Geometry check sheet. Reference: the model listing, model coordinates, mm. Face numbers are marked on the shaded views. A direction names the side the tool comes from. Coordinates: 2 decimals unless noted, no trailing zeros. Loops run counter-clockwise (first coordinate to the right, second up) from the corner with the lowest first, then second, coordinate; pieces in that order, holes last. Notation, with made-up numbers: (77, 41) - (109, 41) arc R25 cw to (109, 65) - close; hole circle Ø10 at (85.25, 3). An arc over 180 degrees is marked (long way). Write each question's results on one line, items separated by ' | '. Start each with the question number.
(1) Sectioned sample at C-C (y = 11.5). Enter the section's corners in (x, z), plus the area to 4 significant figures.
(2) Sectioned sample at D-D (x = -5.5). Enter the section's corners in (y, z), plus the area to 3 significant figures.
(3) Sectioned sample at B-B (z = 0). Enter the section's corners in (x, y), plus the area to 4 significant figures.
(4) Access from +Z, -Z, +X, -X, +Y, -Y to the whole of each face (thin tool, end or side, straight path). Record for the marked faces 4, 5 and 6.
(5) Go/stop test with flat-tipped pins: pin 1 Ø7.5 at (x, z) = (-3, 1.5) entering from -Y; pin 2 Ø4.5 at (x, z) = (0, 32.5) entering from -Y. Record where each tip stops, or that it passes through.
(6) Mould release check, pull along Z, two halves, no side actions. Record for the marked faces 1, 2 and 3: pulls with the +Z half, pulls with the -Z half, needs draft (parallel to the pull), parting line crosses it, or undercut.
(7) Sectioned sample at A-A (y = -34.5). Enter the section's corners in (x, z).
(8) Material ranges on probe 1 along Y at (x, z) = (6.2, 0); probe 2 along X at (y, z) = (-37, -20); probe 3 along Y at (x, z) = (-3.5, 0), recorded low to high.
from build123d import *

# Parameters (mm, degrees)
SKETCH1_R             = 27.5
BOSS_EXTRUDE2_DEPTH   = 7.5
M6_TAPPED_HOLE1_D     = 5
M6_TAPPED_HOLE1_DEPTH = 17
M6_TAPPED_HOLE1_TIP   = 1.502151548
BOSS_EXTRUDE3_START   = -2
SKETCH5_R             = 27.5
SKETCH5_R_2           = 26
BOSS_EXTRUDE3_DEPTH   = 2
CHAMFER1_SIZE         = 5
SKETCH4_R             = 2.5
CUT_EXTRUDE1_DEPTH    = 15
CHAMFER2_SIZE         = 1
CHAMFER3_SIZE         = 0.5


with BuildPart() as part:
    # Sketch1 → Boss-Extrude2 (new, symmetric)
    with BuildSketch(Plane(origin=(0, 0, 0), x_dir=(0, 0, -1), z_dir=(1, 0, 0))):
        with BuildLine():
            Line((-37.5, -42.5), (-12.5, -42.5))
            Line((-12.5, -42.5), (-12.5, -32.5))
            ThreePointArc((-12.5, -32.5), (-11.035533906, -28.964466094), (-7.5, -27.5))
            Line((-7.5, -27.5), (7.5, -27.5))
            ThreePointArc((7.5, -27.5), (11.035533906, -28.964466094), (12.5, -32.5))
            Line((12.5, -32.5), (12.5, -42.5))
            Line((12.5, -42.5), (37.5, -42.5))
            Line((37.5, -42.5), (37.5, 42.5))
            Line((37.5, 42.5), (-37.5, 42.5))
            Line((-37.5, 42.5), (-37.5, -42.5))
        make_face()
        with Locations((0, 11.5)):
            Circle(SKETCH1_R, mode=Mode.SUBTRACT)
    extrude(amount=BOSS_EXTRUDE2_DEPTH, both=True)

    # M6 Tapped Hole1
    with Locations(Plane(origin=(0, -42.5, 0), x_dir=(-1, 0, 0), z_dir=(0, -1, 0))):
        with Locations((0, -32.5), (0, 32.5)):
            Hole(M6_TAPPED_HOLE1_D / 2, depth=M6_TAPPED_HOLE1_DEPTH)
            with Locations((0, 0, -(M6_TAPPED_HOLE1_DEPTH + M6_TAPPED_HOLE1_TIP / 2))):  # 118° drill point
                Cone(0, M6_TAPPED_HOLE1_D / 2, M6_TAPPED_HOLE1_TIP, mode=Mode.SUBTRACT)

    # Sketch5 → Boss-Extrude3 (add)
    with BuildSketch(Plane(origin=(7.5, 0, 0), x_dir=(0, 0, -1), z_dir=(1, 0, 0)).offset(BOSS_EXTRUDE3_START)):
        with Locations((0, 11.5)):
            Circle(SKETCH5_R)
        with Locations((0, 11.5)):
            Circle(SKETCH5_R_2, mode=Mode.SUBTRACT)
    extrude(amount=BOSS_EXTRUDE3_DEPTH)

    # Chamfer1
    chamfer1_edges = [part.edges().sort_by_distance(p)[0] for p in [
        (0, 42.5, 37.5),
        (0, 42.5, -37.5),
    ]]
    chamfer(chamfer1_edges, length=CHAMFER1_SIZE)

    # Sketch4 → Cut-Extrude1 (cut)
    with BuildSketch(Plane.XZ.offset(42.5)):
        with Locations(Location((0, -20, 0), (0, 0, 270))):
            Circle(SKETCH4_R)
        with BuildLine():
            Line((2.5, 20.5), (2.5, 19.5))
            ThreePointArc((2.5, 19.5), (0, 17), (-2.5, 19.5))
            Line((-2.5, 19.5), (-2.5, 20.5))
            ThreePointArc((-2.5, 20.5), (0, 23), (2.5, 20.5))
        make_face()
    extrude(amount=-CUT_EXTRUDE1_DEPTH, mode=Mode.SUBTRACT)

    # Chamfer2
    chamfer2_edges = [part.edges().sort_by_distance(p)[0] for p in [
        (0, -42.5, -12.5),
        (0, -42.5, 12.5),
    ]]
    chamfer(chamfer2_edges, length=CHAMFER2_SIZE)

    # Chamfer3
    chamfer3_edges = [part.edges().sort_by_distance(p)[0] for p in [
        (-7.5, 11.5, 27.5),
        (7.5, 11.5, 26),
    ]]
    chamfer(chamfer3_edges, length=CHAMFER3_SIZE)


solid = part.part
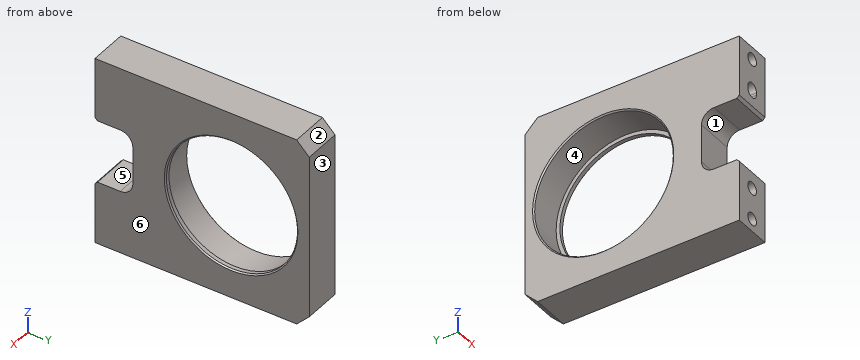
Outcome:
1) outline: (-7.5, -37.5) - (7.5, -37.5) - (7.5, -26.5) - (7, -26) - (5.5, -26) - (5.5, -27.5) - (-7, -27.5) - (-7.5, -28) - close; (-7.5, 28) - (-7, 27.5) - (5.5, 27.5) - (5.5, 26) - (7, 26) - (7.5, 26.5) - (7.5, 37.5) - (-7.5, 37.5) - close | area: 305.5 mm2
2) outline: (-42.5, -37.5) - (37.5, -37.5) - (42.5, -32.5) - (42.5, 32.5) - (37.5, 37.5) - (-42.5, 37.5) - (-42.5, 13.5) - (-41.5, 12.5) - (-32.5, 12.5) arc R5 cw to (-27.5, 7.5) - (-27.5, -7.5) arc R5 cw to (-32.5, -12.5) - (-41.5, -12.5) - (-42.5, -13.5) - close; hole circle Ø55 at (11.5, 0) | area: 3,610 mm2
3) outline: (-7.5, -27.5) - (7.5, -27.5) - (7.5, -15) - (7, -14.5) - (5.5, -14.5) - (5.5, -16) - (-7, -16) - (-7.5, -16.5) - close; (-7.5, 39.5) - (-7, 39) - (5.5, 39) - (5.5, 37.5) - (7, 37.5) - (7.5, 38) - (7.5, 42.5) - (-7.5, 42.5) - close | area: 230.5 mm2
4) face 4: -X | face 5: +X, -X, -Y | face 6: +Z, -Z, +X, +Y, -Y
5) pin 1: stops at y = -27.5 | pin 2: stops at y = -25.35
6) face 1: undercut | face 2: pulls with the +Z half | face 3: needs draft
7) outline: (-7.5, -37.5) - (7.5, -37.5) - (7.5, -12.5) - (-7.5, -12.5) - close; (-7.5, 12.5) - (7.5, 12.5) - (7.5, 37.5) - (-7.5, 37.5) - close; hole circle Ø5 at (0, -32.5); hole circle Ø5 at (0, -20); hole (-2.5, 19.5) arc R2.5 ccw to (2.5, 19.5) - (2.5, 20.5) arc R2.5 ccw to (-2.5, 20.5) - close; hole circle Ø5 at (0, 32.5)
8) probe 1: y = -27.5 to -14.5, 37.5 to 42.5 | probe 2: x = -7.5 to -2.5, 2.5 to 7.5 | probe 3: y = -27.5 to -16, 39 to 42.5
